Could you check a few things on this model? Use its own coordinates, in mm. Give positions to 0.01 mm unless a question says otherwise; leave off trailing zeros. Loops run counter-clockwise (first coordinate to the right, second up) from the corner with the lowest first, then second, coordinate; pieces in that order, holes last. Notation, with made-up numbers: M 22.5,82 L 52.5,82 A20 ccw 52.5,114 Z; hole C 26.5,-32.5 d7. An arc over 180 degrees is marked long. Return JSON: item names as keys, results as strings. Group by question number.
1. Please list where these lines run through material, in increasing order: line 1 (X direction, y = 13, z = 5.5); line 2 (Y direction, x = 50.5, z = 0); line 3 (X direction, y = 14, z = 7).
2. If we mould it in two halves opening along X, with no side actions, what happens to faces 1 (the cylindrical face through (49.01, -3.03, -13.67)), 2 (the flat face through (0, 0, 0)), 3 (the cylindrical face through (2.54, -0.88, 19.98)), 4 (the flat face through (79, 0, 0))? For each: +X half, -X half, draft (parallel to the pull), parting line (faces both ways), or undercut.
3. If we section it at A-A (y = 0): Write out the boundary of the cut face in (x, z), plus the area to 3 significant figures.
4. For pin 1 (3 mm diameter, centred on x = 22, z = -13, fed in from +Y); pin 2 (2 mm diameter, centred on x = 21.5, y = 7.5, fed in from +Z); pin 3 (4 mm diameter, centred on x = 14.5, y = -14, fed in from +Z), each with a flat end and sliding along its axis, tell me the tip position at first contact or that it passes through.
```python
from build123d import *

# Parameters (mm, degrees)
CUT_EXTRUDE_START   = -29
SKETCH_3_R          = 15
SKETCH_3_R_2        = 14
CUT_EXTRUDE_1_DEPTH = 2


with BuildPart() as part:
    # 草图1 → 旋转1 (revolve)
    with BuildSketch(Plane.XY, mode=Mode.PRIVATE) as revolve_1_sk:
        Polygon((0, 0), (0, 20), (5, 20), (5, 16.5), (20, 16.5), (20, 15), (79, 15), (79, 0), align=None)
    revolve(revolve_1_sk.sketch.rotate(Axis((79, 0, 0), (-1, 0, 0)), 90), axis=Axis((79, 0, 0), (-1, 0, 0)))

    # 草图3 → 切除-拉伸1 (cut)
    with BuildSketch(Plane(origin=(79, 0, 0), x_dir=(0, 0, -1), z_dir=(1, 0, 0)).offset(CUT_EXTRUDE_START)):
        Circle(SKETCH_3_R)
        with Locations(Location((0, 0, 0), (0, 0, 90))):
            Circle(SKETCH_3_R_2, mode=Mode.SUBTRACT)
    extrude(amount=-CUT_EXTRUDE_1_DEPTH, mode=Mode.SUBTRACT)


solid = part.part
```
Answer:
{
 "1": {"line 1": "x = 0 to 48, 50 to 79", "line 2": "y = -15 to 15", "line 3": "x = 0 to 20"},
 "2": {"face 1": "undercut", "face 2": "-X half", "face 3": "draft", "face 4": "+X half"},
 "3": {"outline": "M 0,-20 L 5,-20 L 5,-16.5 L 20,-16.5 L 20,-15 L 48,-15 L 48,-14 L 50,-14 L 50,-15 L 79,-15 L 79,15 L 50,15 L 50,14 L 48,14 L 48,15 L 20,15 L 20,16.5 L 5,16.5 L 5,20 L 0,20 Z", "area": "2,460 mm²"},
 "4": {"pin 1": "stops at y = 9.63", "pin 2": "stops at z = 13.52", "pin 3": "stops at z = 11.32"}
}
